```python
from build123d import *

# Parameters (mm, degrees)
EXTRUDE_1_DEPTH     = 748.75
CUT_EXTRUDE_2_DEPTH = 10
CUT_EXTRUDE_3_DEPTH = 752.482909092
SKETCH_6_R          = 1.65
CUT_EXTRUDE_4_DEPTH = 10
SKETCH_7_R          = 2.1
CUT_EXTRUDE_5_DEPTH = 10


with BuildPart() as part:
    # 草图1 → 拉伸-薄壁1 (new, symmetric)
    with BuildSketch(Plane.XY):
        with BuildLine():
            Line((-36, 25), (36, 25))
            ThreePointArc((36, 25), (38.828427125, 23.828427125), (40, 21))
            Line((40, 21), (40, -21))
            ThreePointArc((40, -21), (38.828427125, -23.828427125), (36, -25))
            Line((36, -25), (-36, -25))
            ThreePointArc((-36, -25), (-38.828427125, -23.828427125), (-40, -21))
            Line((-40, -21), (-40, 21))
            ThreePointArc((-40, 21), (-38.828427125, 23.828427125), (-36, 25))
        make_face()
        with BuildLine():
            Line((-36, 22), (36, 22))
            ThreePointArc((36, 22), (36.707106781, 21.707106781), (37, 21))
            Line((37, 21), (37, -21))
            ThreePointArc((37, -21), (36.707106781, -21.707106781), (36, -22))
            Line((36, -22), (-36, -22))
            ThreePointArc((-36, -22), (-36.707106781, -21.707106781), (-37, -21))
            Line((-37, -21), (-37, 21))
            ThreePointArc((-37, 21), (-36.707106781, 21.707106781), (-36, 22))
        make_face(mode=Mode.SUBTRACT)
    extrude(amount=EXTRUDE_1_DEPTH, both=True)

    # 草图4 → 切除-拉伸2 (cut)
    with BuildSketch(Plane.XZ.offset(25)):
        with BuildLine():
            Line((23, 91.25), (23, 111.25))
            ThreePointArc((23, 111.25), (30, 118.25), (37, 111.25))
            Line((37, 111.25), (37, 91.25))
            ThreePointArc((37, 91.25), (30, 84.25), (23, 91.25))
        make_face()
        with BuildLine():
            Line((23, 1.25), (23, 21.25))
            ThreePointArc((23, 21.25), (30, 28.25), (37, 21.25))
            Line((37, 21.25), (37, 1.25))
            ThreePointArc((37, 1.25), (30, -5.75), (23, 1.25))
        make_face()
    extrude(amount=-CUT_EXTRUDE_2_DEPTH, mode=Mode.SUBTRACT)

    # 草图5 → 切除-拉伸3 (cut, through all)
    with BuildSketch(Plane.XZ.offset(25)):
        with BuildLine():
            Line((-10, 26.25), (10, 26.25))
            ThreePointArc((10, 26.25), (13.535533906, 27.714466094), (15, 31.25))
            Line((15, 31.25), (15, 81.25))
            ThreePointArc((15, 81.25), (13.535533906, 84.785533906), (10, 86.25))
            Line((10, 86.25), (-10, 86.25))
            ThreePointArc((-10, 86.25), (-13.535533906, 84.785533906), (-15, 81.25))
            Line((-15, 81.25), (-15, 31.25))
            ThreePointArc((-15, 31.25), (-13.535533906, 27.714466094), (-10, 26.25))
        make_face()
    extrude(amount=-CUT_EXTRUDE_3_DEPTH, mode=Mode.SUBTRACT)

    # 草图6 → 切除-拉伸4 (cut)
    with BuildSketch(Plane(origin=(0, 25, 0), x_dir=(1, 0, 0), z_dir=(0, 1, 0))):
        with Locations(Location((-21.5, -150, 0), (0, 0, 270))):
            Circle(SKETCH_6_R)
        with Locations(Location((-21.5, -193, 0), (0, 0, 270))):
            Circle(SKETCH_6_R)
        with Locations(Location((21.5, -150, 0), (0, 0, 270))):
            Circle(SKETCH_6_R)
        with Locations(Location((21.5, -193, 0), (0, 0, 270))):
            Circle(SKETCH_6_R)
    extrude(amount=-CUT_EXTRUDE_4_DEPTH, mode=Mode.SUBTRACT)

    # 草图7 → 切除-拉伸5 (cut)
    with BuildSketch(Plane.ZY.offset(40)):
        with Locations(Location((108.75, 11, 0), (0, 0, 270))):
            Circle(SKETCH_7_R)
        with Locations(Location((215.75, 11, 0), (0, 0, 270))):
            Circle(SKETCH_7_R)
    extrude(amount=-CUT_EXTRUDE_5_DEPTH, mode=Mode.SUBTRACT)


solid = part.part
```
Could you check a few things on this model? Use its own coordinates, in mm. A direction names the side the tool comes from. Coordinates: 2 decimals unless noted, no trailing zeros. Loops run counter-clockwise (first coordinate to the right, second up) from the corner with the lowest first, then second, coordinate; pieces in that order, holes last. Notation, with made-up numbers: M -5,86.5 L 18,86.5 A33 cw 18,116.5 Z; hole C -22.5,-33.5 d1. An arc over 180 degrees is marked long. Put each result on its own line as item: value. Start each with the question number.
(1) For faces 1 (the face through (-37, 0, 10)), 2 (the face through (-2.8, 22.3, -748.75)), which set-ups out of +Z, -Z, +X, -X, +Y, -Y let a thin tool reach every point of the face, with its end or its side?
(2) I need wall thicknesses on line 1 (Z direction, x = 21, y = 23); line 2 (Z direction, x = -37.7, y = 11); line 3 (X direction, y = -12, z = 451). Which ranges of each line are inside material? Lowest first, please. Write a range as from..to.
(3) Suppose I cut it at B-B on z = 581. Please give me the cut outline in (x, y).
(4) Suppose I cut it at A-A on y = -12.5. Please give me the cut outline in (x, z).
(5) Thinking about a two-plate mould opening in Y: for faces 3 (the face through (1, -25, 10)), 4 (the face through (40, 0, 10)), 5 (the face through (-1, 22, 10)), which applies, pulls with the +Y half, pulls with the -Y half, needs draft (parallel to the pull), parting line crosses it, or undercut?
(6) Will these pins go through, and if not, where does the flat tip stop? P1, Ø3.5, axis at y = 24, z = 63, coming from the +X side; P2, Ø0.9, axis at y = -24, z = 68.5, coming from the -X side; P3, Ø3.5, axis at y = -23.5, z = 63.5, coming from the +X side.
Solutions:
1. face 1: +Z, -Z
1. face 2: -Z, +X, -X, +Y, -Y
2. line 1: z = -748.75..148.43, 151.57..191.43, 194.57..748.75
2. line 2: z = -748.75..106.65, 110.85..213.65, 217.85..748.75
2. line 3: x = -40..-37, 37..40
3. outline: M -40,-21 A4 ccw -36,-25 L 36,-25 A4 ccw 40,-21 L 40,21 A4 ccw 36,25 L -36,25 A4 ccw -40,21 Z; hole M -37,-21 A1 ccw -36,-22 L 36,-22 A1 ccw 37,-21 L 37,21 A1 ccw 36,22 L -36,22 A1 ccw -37,21 Z
4. outline: M -40,-748.75 L -37,-748.75 L -37,748.75 L -40,748.75 Z; M 37,-748.75 L 40,-748.75 L 40,748.75 L 37,748.75 Z
5. face 3: pulls with the -Y half
5. face 4: needs draft
5. face 5: undercut
6. P1: stops at x = 39.8
6. P2: stops at x = -39.08
6. P3: stops at x = 39.93
